```python
from build123d import *

# Parameters (mm, degrees)
SKETCH_1_W             = 40
SKETCH_1_H             = 7
EXTRUDE_1_DEPTH        = 21.5
HOLE_WIZARD_M3_1_D     = 2.5
HOLE_WIZARD_M3_1_DEPTH = 7.5
HOLE_WIZARD_M3_1_TIP   = 0.751075774
SKETCH_4_W             = 4
SKETCH_4_H             = 4
CUT_EXTRUDE_1_DEPTH    = 46.546679352
MM_1_D                 = 2


with BuildPart() as part:
    # 草图1 → 凸台-拉伸1 (new body)
    with BuildSketch(Plane.XY):
        Rectangle(SKETCH_1_W, SKETCH_1_H)
    extrude(amount=EXTRUDE_1_DEPTH)

    # M3 螺纹孔1
    with Locations(Plane.XY.offset(21.5)):
        with Locations((-15, 0), (0, 0), (15, 0)):
            Hole(HOLE_WIZARD_M3_1_D / 2, depth=HOLE_WIZARD_M3_1_DEPTH)
            with Locations((0, 0, -(HOLE_WIZARD_M3_1_DEPTH + HOLE_WIZARD_M3_1_TIP / 2))):  # 118° drill point
                Cone(0, HOLE_WIZARD_M3_1_D / 2, HOLE_WIZARD_M3_1_TIP, mode=Mode.SUBTRACT)

    # 草图4 → 切除-拉伸1 (cut, through all)
    with BuildSketch(Plane(origin=(20, 0, 0), x_dir=(0, 0, -1), z_dir=(1, 0, 0))):
        with Locations((-2, 0)):
            Rectangle(SKETCH_4_W, SKETCH_4_H)
    extrude(amount=-CUT_EXTRUDE_1_DEPTH, mode=Mode.SUBTRACT)

    # 大小mm 暗销孔1 (through all)
    with Locations(Plane(origin=(0, 3.5, 0), x_dir=(1, 0, 0), z_dir=(0, 1, 0))):
        with Locations((-15, -2), (0, -2), (15, -2)):
            Hole(MM_1_D / 2)


solid = part.part
```
The listing builds one solid part. Answer for the finished solid, in the listing's coordinates (mm). A direction names the side the tool comes from. Round coordinates to 2 decimals unless told otherwise and drop trailing zeros. Loops run counter-clockwise (first coordinate to the right, second up) from the corner with the lowest first, then second, coordinate; pieces in that order, holes last.
Q1. For a pull along Y with two mould halves and no side action, classify faces 1 (the face through (0, 3.5, 11)), 2 (the face through (0, 2, 21.5)), 3 (the face through (0.27, -1.22, 17.7)) as released by +Y, released by -Y, zero draft, split by the parting line, or undercut.
Q2. Section C-C, the plane x = 11.5 is taken. Determine the outline of the cut face in (y, z), then the cut area to 4 significant figures.
Q3. Find the intervals of material crossed by line 1 (X direction, y = 0, z = 18); line 2 (Z direction, x = -15, y = -2.5); line 3 (Y direction, x = 12.5, z = 2), in increasing order.
Q4. Section B-B, the plane z = 19.5 is taken. Determine the outline of the cut face in (x, y), then the cut area to 3 significant figures.
Q5. Which of the six approach directions +Z, -Z, +X, -X, +Y, -Y give full straight-line access (tool end or side, diameter ignored) to faces 4 (the face through (-13.75, 0.05, 17.7)), 5 (the face through (0, -3.5, 11)), 6 (the face through (0.3, -2, 3.4))?
Q6. Section A-A, the plane z = 2 is taken. Count the separate pieces of the cut face and the enclosed holes in it, then the cut area to 3 significant figures.
Q7. Given pin 1 Ø3 at (x, y) = (15, 0) entering from -Z; pin 2 Ø1.6 at (x, z) = (-15, 2) entering from -Y, each flat-ended and moving along its own axis, determine where each tip first touches the part or whether it passes through.
Completed:
1. face 1: released by +Y
1. face 2: zero draft
1. face 3: undercut
2. outline: (-3.5, 0) - (-2, 0) - (-2, 4) - (2, 4) - (2, 0) - (3.5, 0) - (3.5, 21.5) - (-3.5, 21.5) - close
2. area: 134.5 mm2
3. line 1: x = -20 to -16.25, -13.75 to -1.25, 1.25 to 13.75, 16.25 to 20
3. line 2: z = 0 to 1, 3 to 21.5
3. line 3: y = -3.5 to -2, 2 to 3.5
4. outline: (-20, -3.5) - (20, -3.5) - (20, 3.5) - (-20, 3.5) - close; hole circle Ø2.5 at (-15, 0); hole circle Ø2.5 at (0, 0); hole circle Ø2.5 at (15, 0)
4. area: 265 mm2
5. face 4: +Z
5. face 5: +Z, -Z, +X, -X, -Y
5. face 6: -Z, +X, -X
6. separate pieces: 8
6. enclosed holes: 0
6. area: 102 mm2
7. pin 1: stops at z = 4
7. pin 2: passes through
